```python
from build123d import *


with BuildPart() as part:
    # 草图1 → 旋转1 (revolve)
    with BuildSketch(Plane.XY, mode=Mode.PRIVATE) as revolve_1_sk:
        Polygon((20.5, -6), (18.5, -2.5), (18.5, 2.5), (20.5, 6), (20.5, 7), (11, 7), (11, 1), (8, 1), (8, -1), (11, -1), (11, -7), (20.5, -7), align=None)
    revolve(revolve_1_sk.sketch.rotate(Axis((0, 20.639192491, 0), (0, -1, 0)), 90), axis=Axis((0, 20.639192491, 0), (0, -1, 0)))


solid = part.part
```
Input: part model. Units: mm. Frame: model coordinates. A direction names the side the tool comes from. Round coordinates to 2 decimals unless told otherwise and drop trailing zeros. Loops run counter-clockwise (first coordinate to the right, second up) from the corner with the lowest first, then second, coordinate; pieces in that order, holes last. Notation, with made-up numbers: M -15.75,39 L 21.25,39 A23 cw 21.25,64 Z; hole C 27.25,42.25 d8. An arc over 180 degrees is marked long. Answer in a Markdown table with one row per item. Add a question column.
1. Mould query, pull axis Y, two halves, no side actions, for faces 5 (the face through (7.852, 6.507, 18.937)), 6 (the face through (9, -7, -9)), 7 (the face through (16.41, 0.04, 8.54)), 8 (the face through (-5.586, -2.67, 17.738)). Classes: released by +Y, released by -Y, zero draft, split by the parting line, or undercut.
2. Contact query for flat-ended pins moving along their axis: pin 1 (3 mm diameter, centred on x = -1.5, z = 7.5, fed in from +Y); pin 2 (4 mm diameter, centred on y = -0.5, z = -9, fed in from +X); pin 3 (2 mm diameter, centred on y = -1, z = 11, fed in from -X). Output: stop coordinate, or through.
3. Section D-D (y = -4.5). Output: boundary loops of the cut face in (x, z), and give its area (3 significant figures).
4. Ray query, probe 1 along X at (y, z) = (2.3, 0); probe 2 along X at (y, z) = (-0.5, 0); probe 3 along Y at (x, z) = (-7.5, -4). Return the intervals inside material, ascending.
5. Set-up query: faces 1 (the face through (10.74, 3.96, -2.38)), 2 (the face through (7.81, -0.01, -1.73)), 3 (the face through (-5.594, 2.719, 17.765)), 4 (the face through (10.74, -4.04, -2.38)). Return all of +Z, -Z, +X, -X, +Y, -Y with unobstructed straight access to the full face (end or side cutting, diameter ignored); none if empty.
6. Section B-B (x = 0). Output: boundary loops of the cut face in (y, z), and give its area (3 significant figures).
7. Section C-C (y = -0.25). Output: boundary loops of the cut face in (x, z), and give its area (3 significant figures).
8. Section A-A (z = 0). Output: boundary loops of the cut face in (x, y), and give its area (3 significant figures).
Values follow:
| question | item | result |
|---|---|---|
| 1 | face 5 | zero draft |
| 1 | face 6 | released by -Y |
| 1 | face 7 | undercut |
| 1 | face 8 | undercut |
| 2 | pin 1 | y = 1 |
| 2 | pin 2 | x = 17.12 |
| 2 | pin 3 | x = -15.56 |
| 3 | outline | C 0,0 d39.29; hole C 0,0 d22 |
| 3 | area | 832 mm^2 |
| 4 | probe 1 | -18.5 to -11, 11 to 18.5 |
| 4 | probe 2 | -18.5 to -8, 8 to 18.5 |
| 4 | probe 3 | -1 to 1 |
| 5 | face 1 | +Y |
| 5 | face 2 | +Y, -Y |
| 5 | face 3 | none |
| 5 | face 4 | -Y |
| 6 | outline | M -7,-20.5 L -6,-20.5 L -2.5,-18.5 L 2.5,-18.5 L 6,-20.5 L 7,-20.5 L 7,-11 L 1,-11 L 1,-8 L -1,-8 L -1,-11 L -7,-11 Z; M -7,11 L -1,11 L -1,8 L 1,8 L 1,11 L 7,11 L 7,20.5 L 6,20.5 L 2.5,18.5 L -2.5,18.5 L -6,20.5 L -7,20.5 Z |
| 6 | area | 244 mm^2 |
| 7 | outline | C 0,0 d37; hole C 0,0 d16 |
| 7 | area | 874 mm^2 |
| 8 | outline | M -20.5,-7 L -11,-7 L -11,-1 L -8,-1 L -8,1 L -11,1 L -11,7 L -20.5,7 L -20.5,6 L -18.5,2.5 L -18.5,-2.5 L -20.5,-6 Z; M 8,-1 L 11,-1 L 11,-7 L 20.5,-7 L 20.5,-6 L 18.5,-2.5 L 18.5,2.5 L 20.5,6 L 20.5,7 L 11,7 L 11,1 L 8,1 Z |
| 8 | area | 244 mm^2 |
